Input: part model. Units: mm. Frame: model coordinates. A direction names the side the tool comes from. Round coordinates to 2 decimals unless told otherwise and drop trailing zeros. Loops run counter-clockwise (first coordinate to the right, second up) from the corner with the lowest first, then second, coordinate; pieces in that order, holes last. Notation, with made-up numbers: (56, 6) -> (78, 6) arc R21 ccw to (78, 21) -> close; hole circle Ø6 at (33, 22.5). An arc over 180 degrees is marked (long way). One line per question, with ' | ' between items. Start each with the question number.
Q1. Material intervals for L1, parallel to Z at x = -8.5, y = -14.5; L2, parallel to Y at x = 0, z = 263.5; L3, parallel to X at y = 1.5, z = 74, sorted ascending.
Q2. Cut plane C-C on z = 82. Return loops of the section in (x, y), and give its area (3 significant figures).
Q3. Access query for faces 1 (the face through (11.2, 6.1, -325)), 2 (the face through (11.923, 3.755, 343.98)), 3 (the face through (0, 0, 365)). Directions: +Z, -Z, +X, -X, +Y, -Y. A direction counts if a zero-diameter tool reaches every point of the face in a straight line with its end or side. Return the directions, or none.
Q4. Cut plane A-A on y = 0. Return loops of the section in (x, z), and give its area (3 significant figures).
Q5. Contact query for flat-ended pins moving along their axis: P1, Ø6, axis at x = 21.5, y = 5, coming from the +Z side; P2, Ø3, axis at x = -13.5, y = 20, coming from the -Z side; P3, Ø10, axis at x = -13.5, z = 170, coming from the -Y side. Output: stop coordinate, or through.
from build123d import *

# Parameters (mm, degrees)
SKETCH1_R           = 27.5
BOSS_EXTRUDE1_DEPTH = 325
SKETCH2_R           = 12.5
BOSS_EXTRUDE2_DEPTH = 40
CHAMFER1_SIZE       = 1.5


with BuildPart() as part:
    # Sketch1 → Boss-Extrude1 (new, symmetric)
    with BuildSketch(Plane.XY):
        Circle(SKETCH1_R)
    extrude(amount=BOSS_EXTRUDE1_DEPTH, both=True)

    # Sketch2 → Boss-Extrude2 (add)
    with BuildSketch(Plane.XY.offset(325)):
        Circle(SKETCH2_R)
    boss_extrude2 = extrude(amount=BOSS_EXTRUDE2_DEPTH)

    # Mirror1: Boss-Extrude2 across plane
    add(boss_extrude2.mirror(Plane.XY))

    # Chamfer1
    chamfer1_edges = [part.edges().sort_by_distance(p)[0] for p in [
        (-12.5, 0, -365),
        (-27.5, 0, -325),
        (-27.5, 0, 325),
        (-12.5, 0, 365),
    ]]
    chamfer(chamfer1_edges, length=CHAMFER1_SIZE)


solid = part.part
Results:
1) L1: -325 to 325 | L2: -27.5 to 27.5 | L3: -27.46 to 27.46
2) outline: circle Ø55 at (0, 0) | area: 2,380 mm^2
3) face 1: -Z | face 2: +Z | face 3: +Z, +X, -X, +Y, -Y
4) outline: (-27.5, -323.5) -> (-26, -325) -> (-12.5, -325) -> (-12.5, -363.5) -> (-11, -365) -> (11, -365) -> (12.5, -363.5) -> (12.5, -325) -> (26, -325) -> (27.5, -323.5) -> (27.5, 323.5) -> (26, 325) -> (12.5, 325) -> (12.5, 363.5) -> (11, 365) -> (-11, 365) -> (-12.5, 363.5) -> (-12.5, 325) -> (-26, 325) -> (-27.5, 323.5) -> close | area: 37,700 mm^2
5) P1: z = 325 | P2: z = -325 | P3: y = -26.15
